from build123d import *

# Parameters (mm, degrees)
SKETCH1_W             = 50
SKETCH1_H             = 56
SKETCH1_R             = 6
BOSS_EXTRUDE1_DEPTH   = 8
SKETCH2_W             = 50
SKETCH2_H             = 35
BOSS_EXTRUDE2_DEPTH   = 12
SKETCH3_W             = 20
SKETCH3_H             = 35
CUT_EXTRUDE1_DEPTH    = 8
SKETCH4_W             = 6
SKETCH4_H             = 44
CUT_EXTRUDE2_DEPTH    = 60
CHAMFER2_SIZE         = 5
SKETCH5_W             = 6
SKETCH5_H             = 20
CUT_EXTRUDE3_DEPTH    = 60
M4_TAPPED_HOLE1_D     = 3.3
FILLET1_R             = 3
SKETCH9_R             = 1.75
CUT_EXTRUDE4_DEPTH    = 10
SKETCH10_R            = 1.75
CUT_EXTRUDE5_DEPTH    = 10
M3_TAPPED_HOLE1_D     = 2.5
M3_TAPPED_HOLE1_DEPTH = 7.5
M3_TAPPED_HOLE1_TIP   = 0.751075774
CHAMFER3_SIZE         = 1


with BuildPart() as part:
    # Sketch1 → Boss-Extrude1 (new body)
    with BuildSketch(Plane.XY):
        Rectangle(SKETCH1_W, SKETCH1_H)
        with Locations((0, 5.2)):
            Circle(SKETCH1_R, mode=Mode.SUBTRACT)
    extrude(amount=BOSS_EXTRUDE1_DEPTH)

    # Sketch2 → Boss-Extrude2 (add)
    with BuildSketch(Plane.XZ.offset(28)):
        with Locations((0, 17.5)):
            Rectangle(SKETCH2_W, SKETCH2_H)
    extrude(amount=-BOSS_EXTRUDE2_DEPTH)

    # Sketch3 → Cut-Extrude1 (cut)
    with BuildSketch(Plane.XZ.offset(28)):
        with Locations((0, 17.5)):
            Rectangle(SKETCH3_W, SKETCH3_H)
    extrude(amount=-CUT_EXTRUDE1_DEPTH, mode=Mode.SUBTRACT)

    # Sketch4 → Cut-Extrude2 (cut)
    with BuildSketch(Plane.XY.offset(35)):
        with Locations((-22, 6)):
            Rectangle(SKETCH4_W, SKETCH4_H)
        with Locations((22, 6)):
            Rectangle(SKETCH4_W, SKETCH4_H)
    extrude(amount=-CUT_EXTRUDE2_DEPTH, mode=Mode.SUBTRACT)

    # Chamfer2
    chamfer2_edges = [part.edges().sort_by_distance(p)[0] for p in [
        (-19, 28, 4),
        (19, 28, 4),
    ]]
    chamfer(chamfer2_edges, length=CHAMFER2_SIZE)

    # Sketch5 → Cut-Extrude3 (cut)
    with BuildSketch(Plane(origin=(0, 28, 0), x_dir=(1, 0, 0), z_dir=(0, 1, 0))):
        with Locations((-22, -10)):
            Rectangle(SKETCH5_W, SKETCH5_H)
        with Locations((22, -10)):
            Rectangle(SKETCH5_W, SKETCH5_H)
    extrude(amount=-CUT_EXTRUDE3_DEPTH, mode=Mode.SUBTRACT)

    # M4 Tapped Hole1 (through all)
    with Locations(Plane(origin=(0, -28, 0), x_dir=(-1, 0, 0), z_dir=(0, -1, 0))):
        with Locations((20, -27.5), (-20, -27.5)):
            Hole(M4_TAPPED_HOLE1_D / 2)

    # Fillet1
    fillet1_edges = [part.edges().sort_by_distance(p)[0] for p in [
        (-19, -22, 20),
        (19, -22, 20),
    ]]
    fillet(fillet1_edges, radius=FILLET1_R)

    # Sketch9 → Cut-Extrude4 (cut)
    with BuildSketch(Plane(origin=(0, -16, 0), x_dir=(1, 0, 0), z_dir=(0, 1, 0))):
        with Locations(Location((-7.5, -15, 0), (0, 0, 270))):
            Circle(SKETCH9_R)
        with Locations(Location((7.5, -15, 0), (0, 0, 90))):
            Circle(SKETCH9_R)
        with Locations(Location((-7.5, -25, 0), (0, 0, 270))):
            Circle(SKETCH9_R)
        with Locations(Location((7.5, -25, 0), (0, 0, 90))):
            Circle(SKETCH9_R)
    extrude(amount=-CUT_EXTRUDE4_DEPTH, mode=Mode.SUBTRACT)

    # Sketch10 → Cut-Extrude5 (cut)
    with BuildSketch(Plane.XY.offset(8)):
        with Locations((10, 5.2)):
            Circle(SKETCH10_R)
        with Locations((0, 15.2)):
            Circle(SKETCH10_R)
        with Locations((-10, 5.2)):
            Circle(SKETCH10_R)
        with Locations((0, -4.8)):
            Circle(SKETCH10_R)
    extrude(amount=-CUT_EXTRUDE5_DEPTH, mode=Mode.SUBTRACT)

    # M3 Tapped Hole1
    with Locations(Plane(origin=(19, 0, 0), x_dir=(0, 0, -1), z_dir=(1, 0, 0))):
        with Locations((-5, -23)):
            Hole(M3_TAPPED_HOLE1_D / 2, depth=M3_TAPPED_HOLE1_DEPTH)
            with Locations((0, 0, -(M3_TAPPED_HOLE1_DEPTH + M3_TAPPED_HOLE1_TIP / 2))):  # 118° drill point
                Cone(0, M3_TAPPED_HOLE1_D / 2, M3_TAPPED_HOLE1_TIP, mode=Mode.SUBTRACT)

    # Chamfer3
    chamfer3_edges = [part.edges().sort_by_distance(p)[0] for p in [
        (-25, -22, 20),
        (25, -22, 20),
        (-25, -22, 35),
        (25, -22, 35),
    ]]
    chamfer(chamfer3_edges, length=CHAMFER3_SIZE)


solid = part.part
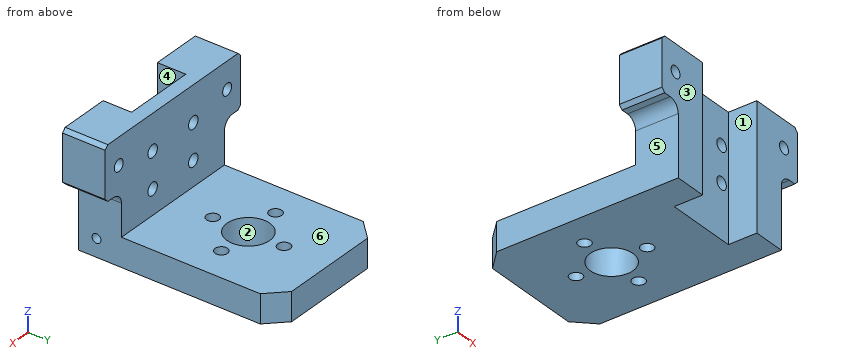
Source: CAD feature listing. Evaluate the final solid. Frame: model axes, mm. Face numbers are marked on the shaded views. A direction names the side the tool comes from. Give positions to 0.01 mm unless a question says otherwise; leave off trailing zeros. Write each loop counter-clockwise with the first axis right and the second up, starting at its lowest first coordinate (ties: lowest second). Pieces come first, ordered by that corner, then holes. Notation, with made-up numbers: M 59,42.25 L 96,42.25 A13 ccw 96,64.25 Z; hole C 1.5,13 d8. An arc over 180 degrees is marked long. Answer as a JSON object with one key per item and string values.
Q1. Cut plane A-A, the plane z = 15. Return the cut outline in (x, y), then the cut area to 3 significant figures.
Geometry check:
{"outline": "M -19,-28 L -10,-28 L -10,-20 L -9.25,-20 L -9.25,-16 L -19,-16 Z; M -5.75,-20 L 5.75,-20 L 5.75,-16 L -5.75,-16 Z; M 9.25,-20 L 10,-20 L 10,-28 L 19,-28 L 19,-16 L 9.25,-16 Z", "area": "268 mm^2"}
Q2. Mould query, pull axis Y, two halves, no side actions, for the marked faces 1, 2 and 3. Classes: +Y half, -Y half, draft (parallel to the pull), parting line (faces both ways), or undercut.
Geometry check:
{"face 1": "draft", "face 2": "undercut", "face 3": "-Y half"}
Q3. Ray query, line 1 along X through (y, z) = (-18, 25); line 2 along X through (y, z) = (-18, 15); line 3 along Y through (x, z) = (-7, 12.5). Return the intervals inside material, ascending.
Geometry check:
{"line 1": "x = -25 to -9.25, -5.75 to 5.75, 9.25 to 25", "line 2": "x = -19 to -9.25, -5.75 to 5.75, 9.25 to 19", "line 3": "y = -20 to -16"}
Q4. Cut plane B-B, the plane y = -4.8. Return the cut outline in (x, z), then the cut area to 3 significant figures.
Geometry check:
{"outline": "M -19,0 L -1.75,0 L -1.75,8 L -19,8 Z; M 1.75,0 L 19,0 L 19,8 L 1.75,8 Z", "area": "276 mm^2"}
Q5. Access query for the marked faces 4, 5 and 6. Directions: +Z, -Z, +X, -X, +Y, -Y. A direction counts if a zero-diameter tool reaches every point of the face in a straight line with its end or side. Return the directions, or none.
Geometry check:
{"face 4": "+Z, -Z, -Y", "face 5": "-Z, -X, +Y, -Y", "face 6": "+Z, +X, -X, +Y"}
Q6. Contact query for flat-ended pins moving along their axis: P1, Ø1, axis at x = 4.5, y = 0, coming from the -Z side; P2, Ø5, axis at x = 4.5, y = 22.5, coming from the +Z side; P3, Ø2.5, axis at x = -20, z = 27.5, coming from the -Y side; P4, Ø4.5, axis at x = 7.5, z = 15, coming from the +Y side. Output: stop coordinate, or through.
Geometry check:
{"P1": "stops at z = 0", "P2": "stops at z = 8", "P3": "passes through", "P4": "stops at y = -16"}
Q7. Cut plane C-C, the plane x = -7.5. Return the cut outline in (y, z), then the cut area to 3 significant figures.
Geometry check:
{"outline": "M -20,0 L 28,0 L 28,8 L -16,8 L -16,13.25 L -20,13.25 Z; M -20,16.75 L -16,16.75 L -16,23.25 L -20,23.25 Z; M -20,26.75 L -16,26.75 L -16,35 L -20,35 Z", "area": "464 mm^2"}
Q8. Cut plane D-D, the plane x = 12.5. Return the cut outline in (y, z), then the cut area to 3 significant figures.
Geometry check:
{"outline": "M -28,0 L 28,0 L 28,8 L -16,8 L -16,35 L -28,35 Z; hole C -23,5 d2.5", "area": "767 mm^2"}
